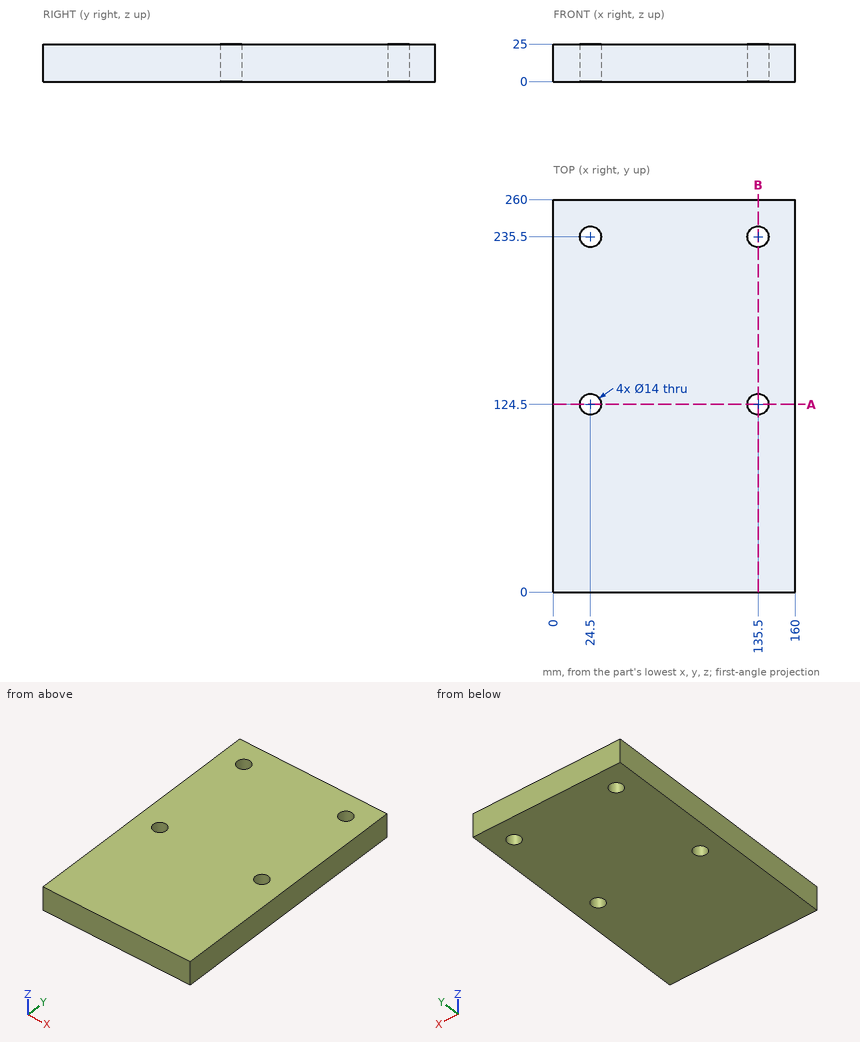
Could you check a few things on this drawing? It's one solid part, dimensions in mm from its lowest x, y, z. Give positions to 0.01 mm unless a question says otherwise; leave off trailing zeros. Write each loop counter-clockwise with the first axis right and the second up, starting at its lowest first coordinate (ties: lowest second). Pieces come first, ordered by that corner, then holes.
(1) If I drill on L1, parallel to Y at x = 24.5, z = 14.5; L2, parallel to Y at x = 129.5, z = 5; L3, parallel to X at y = 230, z = 19, over which ranges is the centre line in solid material (lowest first)?
Output values:
L1: y = 0 to 117.5, 131.5 to 228.5, 242.5 to 260
L2: y = 0 to 120.89, 128.11 to 231.89, 239.11 to 260
L3: x = 0 to 20.17, 28.83 to 131.17, 139.83 to 160
(2) Will this pin go through, and if not, where does the flat tip stop? pin 1 (8.5 mm diameter, centred on x = 24.5, y = 124.5, fed in from -Z).
Output values:
pin 1: passes through
(3) Imagine slicing it at B-B, the plane x = 135.5. Write out the boundary of the cut face in (y, z), and give its area (3 significant figures).
Output values:
outline: (0, 0) - (117.5, 0) - (117.5, 25) - (0, 25) - close; (131.5, 0) - (228.5, 0) - (228.5, 25) - (131.5, 25) - close; (242.5, 0) - (260, 0) - (260, 25) - (242.5, 25) - close
area: 5,800 mm2
(4) Imagine slicing it at A-A, the plane y = 124.5. Write out the boundary of the cut face in (x, z).
Output values:
outline: (0, 0) - (17.5, 0) - (17.5, 25) - (0, 25) - close; (31.5, 0) - (128.5, 0) - (128.5, 25) - (31.5, 25) - close; (142.5, 0) - (160, 0) - (160, 25) - (142.5, 25) - close
